Job drawing, mm, ordinate dimensions from the low corner. One solid piece. A direction names the side the tool comes from. Coordinates: 2 decimals unless noted, no trailing zeros. Loops run counter-clockwise (first coordinate to the right, second up) from the corner with the lowest first, then second, coordinate; pieces in that order, holes last. Notation, with made-up numbers: (-36, 45) - (-31, 45) arc R25 ccw to (-31, 62) - close; hole circle Ø9 at (26, 14). An arc over 180 degrees is marked (long way). Use a Markdown table: item, result. Add a question column.
1. Band-saw the part on B-B, the plane x = 12. Give the cut face in (y, z), plus the area to 3 significant figures.
2. Band-saw the part on C-C, the plane z = 11.75. Give the cut face in (x, y), plus the area to 3 significant figures.
3. 3-axis set-ups, long thin cutter, end or side, ignore diameter. For the marked faces 1 and 2: which of +Z, -Z, +X, -X, +Y, -Y reach the whole face in a straight line?
4. Pull direction Y, two halves, no side cores. Call the marked faces 3, 4 and 5: pulls with the +Y half, pulls with the -Y half, needs draft (parallel to the pull), parting line crosses it, or undercut.
5. Band-saw the part on A-A, the plane y = 12.5. Give the cut face in (x, z).
6. Wall check: probe 1 along Y at (x, z) = (12, 10.5); probe 2 along Z at (x, y) = (32, 3.5); probe 3 along X at (y, z) = (14, 8.75). Give the ranges that are in metal, low to high. Write a range as [from, to].
7. Band-saw the part on D-D, the plane y = 20.25. Give the cut face in (x, z), plus the area to 3 significant figures.
8. Drop a flat-ended pin along its axis: pin 1 (7.5 mm diameter, centred on y = 15, z = 25, fed in from -X). Give the stop position or say it passes through.
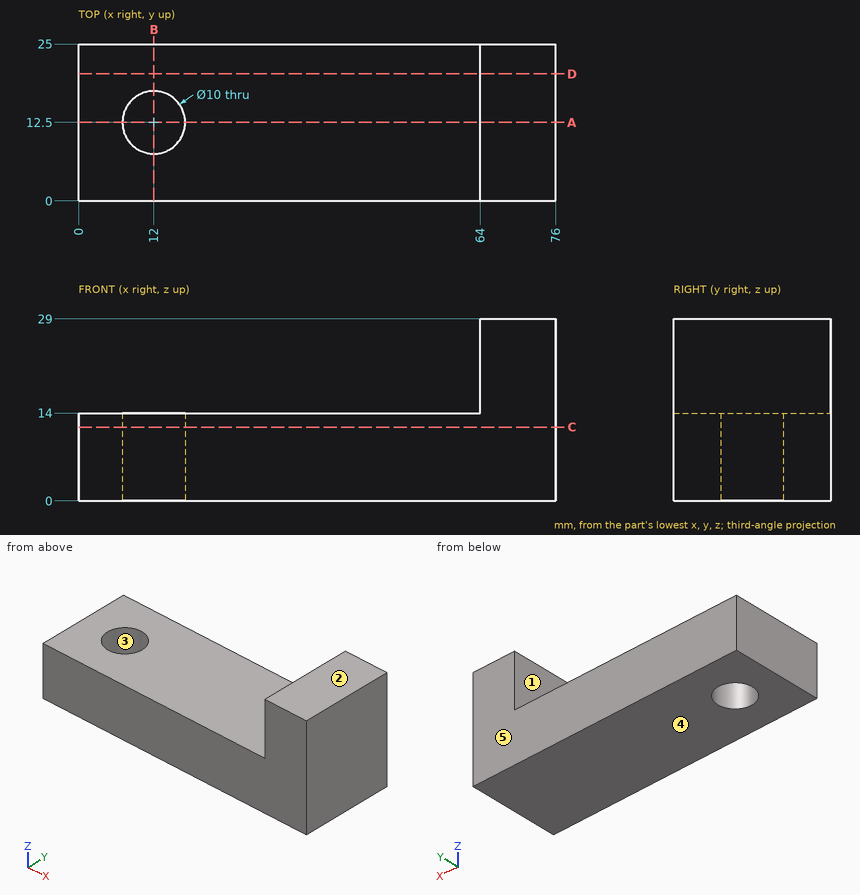
Geometry check:
| question | item | result |
|---|---|---|
| 1 | outline | (0, 0) - (7.5, 0) - (7.5, 14) - (0, 14) - close; (17.5, 0) - (25, 0) - (25, 14) - (17.5, 14) - close |
| 1 | area | 210 mm^2 |
| 2 | outline | (0, 0) - (76, 0) - (76, 25) - (0, 25) - close; hole circle Ø10 at (12, 12.5) |
| 2 | area | 1,820 mm^2 |
| 3 | face 1 | +Z, -X, +Y, -Y |
| 3 | face 2 | +Z, +X, -X, +Y, -Y |
| 4 | face 3 | undercut |
| 4 | face 4 | needs draft |
| 4 | face 5 | pulls with the +Y half |
| 5 | outline | (0, 0) - (7, 0) - (7, 14) - (0, 14) - close; (17, 0) - (76, 0) - (76, 29) - (64, 29) - (64, 14) - (17, 14) - close |
| 6 | probe 1 | y = [0, 7.5], [17.5, 25] |
| 6 | probe 2 | z = [0, 14] |
| 6 | probe 3 | x = [0, 7.23], [16.77, 76] |
| 7 | outline | (0, 0) - (76, 0) - (76, 29) - (64, 29) - (64, 14) - (0, 14) - close |
| 7 | area | 1,240 mm^2 |
| 8 | pin 1 | stops at x = 64 |
